Geometry: final body of the model. Coordinates: model frame, mm. A direction names the side the tool comes from. Give positions to 0.01 mm unless a question says otherwise; leave off trailing zeros. Write each loop counter-clockwise with the first axis right and the second up, starting at its lowest first coordinate (ties: lowest second). Pieces come first, ordered by that corner, then holes. Notation, with made-up numbers: (83, 44.25) -> (130, 44.25) arc R25 cw to (130, 64.25) -> close; hole circle Ø4 at (18.5, 43.25). An arc over 180 degrees is marked (long way). Answer as a JSON object with one key per item and string values.
from build123d import *

# Parameters (mm, degrees)
SKETCH_1_R          = 10
EXTRUDE_1_DEPTH     = 235
CUT_EXTRUDE_START   = 1.3
SKETCH_7_R          = 10
SKETCH_7_R_2        = 9.5
CUT_EXTRUDE_3_DEPTH = 1.3
SKETCH_8_R          = 10
SKETCH_8_R_2        = 9.5
CUT_EXTRUDE_4_DEPTH = 1.3
ZJCQC_DEPTH         = 3.5


with BuildPart() as part:
    # 草图1 → 凸台-拉伸1 (new body)
    with BuildSketch(Plane(origin=(0, 0, 0), x_dir=(1, 0, 0), z_dir=(0, 1, 0))):
        with Locations(Location((0, 0, 0), (0, 0, 90))):
            Circle(SKETCH_1_R)
    extrude(amount=EXTRUDE_1_DEPTH)

    # 草图7 → 切除-拉伸3 (cut)
    with BuildSketch(Plane(origin=(0, 70, 0), x_dir=(-1, 0, 0), z_dir=(0, -1, 0)).offset(CUT_EXTRUDE_START)):
        with Locations(Location((0, 0, 0), (0, 0, 90))):
            Circle(SKETCH_7_R)
        with Locations(Location((0, 0, 0), (0, 0, 90))):
            Circle(SKETCH_7_R_2, mode=Mode.SUBTRACT)
    extrude(amount=-CUT_EXTRUDE_3_DEPTH, mode=Mode.SUBTRACT)

    # 草图8 → 切除-拉伸4 (cut)
    with BuildSketch(Plane(origin=(0, 165, 0), x_dir=(1, 0, 0), z_dir=(0, 1, 0))):
        with Locations(Location((0, 0, 0), (0, 0, 90))):
            Circle(SKETCH_8_R)
        with Locations(Location((0, 0, 0), (0, 0, 90))):
            Circle(SKETCH_8_R_2, mode=Mode.SUBTRACT)
    extrude(amount=CUT_EXTRUDE_4_DEPTH, mode=Mode.SUBTRACT)

    # MyToolsZJC → ZJCQC (cut)
    with BuildSketch(Plane.YX.offset(10)):
        with BuildLine():
            Line((115.5, 3), (119.5, 3))
            ThreePointArc((119.5, 3), (122.5, 0), (119.5, -3))
            Line((119.5, -3), (115.5, -3))
            ThreePointArc((115.5, -3), (112.5, 0), (115.5, 3))
        make_face()
    extrude(amount=-ZJCQC_DEPTH, mode=Mode.SUBTRACT)


solid = part.part
Q1. Material intervals for L1, parallel to X at y = 112, z = 0; L2, parallel to Z at x = 0.5, y = 206.5; L3, parallel to X at y = 151, z = 3, sorted ascending. Write a range as from..to.
Values:
{"L1": "-10..10", "L2": "-9.99..9.99", "L3": "-9.54..9.54"}
Q2. Set-up query: faces 4 (the flat face through (4, 166.3, -9)), 5 (the flat face through (0, 0, 0)). Return all of +Z, -Z, +X, -X, +Y, -Y with unobstructed straight access to the full face (end or side cutting, diameter ignored); none if empty.
Values:
{"face 4": "none", "face 5": "+Z, -Z, +X, -X, -Y"}
Q3. Cut plane A-A (z = 2.5). Return the cut outline in (x, y).
Values:
{"outline": "(-9.68, 0) -> (9.68, 0) -> (9.68, 68.7) -> (9.17, 68.7) -> (9.17, 70) -> (9.68, 70) -> (9.68, 165) -> (9.17, 165) -> (9.17, 166.3) -> (9.68, 166.3) -> (9.68, 235) -> (-9.68, 235) -> (-9.68, 166.3) -> (-9.17, 166.3) -> (-9.17, 165) -> (-9.68, 165) -> (-9.68, 70) -> (-9.17, 70) -> (-9.17, 68.7) -> (-9.68, 68.7) -> close"}
Q4. Mould query, pull axis X, two halves, no side actions, for faces 1 (the flat face through (0, 118, -6.5)), 2 (the cylindrical face through (5.78, 165.64, 7.54)), 3 (the flat face through (-4, 70, -9)). Classes: pulls with the +X half, pulls with the -X half, needs draft (parallel to the pull), parting line crosses it, or undercut.
Values:
{"face 1": "undercut", "face 2": "parting line crosses it", "face 3": "needs draft"}
Q5. First-contact query: P1, Ø1.5, axis at x = -7.5, y = 56, coming from the -Z side; P2, Ø3.5, axis at y = 118, z = -8.5, coming from the +X side; P3, Ø1.8, axis at x = -1.5, y = 118, coming from the -Z side. Flat tips, straight axial feed; report the tip coordinate or a pass-through.
Values:
{"P1": "z = -7.38", "P2": "x = 7.38", "P3": "z = -6.5"}
Q6. Cut plane B-B (y = 92.5). Return the cut outline in (x, z), and give its area (3 significant figures).
Values:
{"outline": "circle Ø20 at (0, 0)", "area": "314 mm²"}
